Build history of the part. All positions in model axes, mm. Face numbers are marked on the shaded views. A direction names the side the tool comes from. Round coordinates to 2 decimals unless told otherwise and drop trailing zeros. Loops run counter-clockwise (first coordinate to the right, second up) from the corner with the lowest first, then second, coordinate; pieces in that order, holes last. Notation, with made-up numbers: (49.5, 10) -> (74.5, 10) arc R24 cw to (74.5, 28) -> close; hole circle Ø5 at (68, 1). An arc over 180 degrees is marked (long way). Put each result on its own line as item: value. Start each with the question number.
Item 1: Tool access for the marked faces 4, 5 and 6: list every direction of +Z, -Z, +X, -X, +Y, -Y with a clear straight run to the whole face (end or side of a thin tool).
Item 2: Flat gauge pins, fed straight in: pin 1 Ø8.5 at (x, z) = (0, 0) entering from +Y; pin 2 Ø3 at (x, z) = (4, 7) entering from +Y; pin 3 Ø1 at (x, z) = (-0.5, -1.5) entering from +Y. Where does each tip first touch, or does it go through?
Item 3: Cut at A-A, the plane y = -28. List the corners of the cut face in (x, z), plus the area to 3 significant figures.
Item 4: Pull direction X, two halves, no side cores. Call the marked faces 1, 2 and 3: +X half, -X half, draft (parallel to the pull), parting line (faces both ways), or undercut.
Item 5: Drill centre lines: probe 1 along X at (y, z) = (-32, 0); probe 2 along Y at (x, z) = (3.25, 5.5); probe 3 along Z at (x, y) = (0, -32.5). Where is each one in solid material? Low to high. Write a range as [from, to].
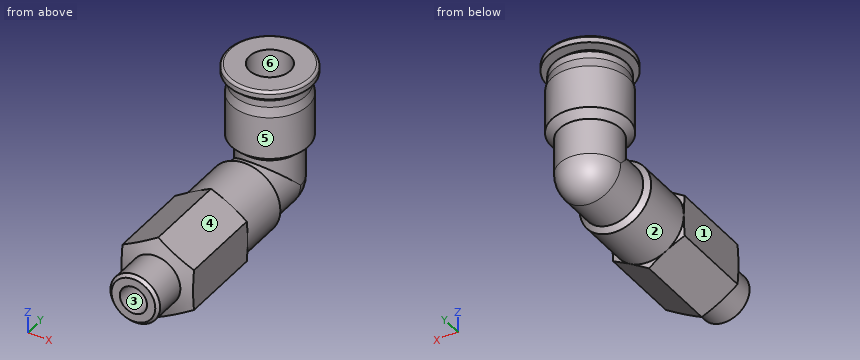
```python
from build123d import *

# Parameters (mm, degrees)
SKETCH_3_R          = 14
CUT_EXTRUDE_1_DEPTH = 21.4
SKETCH_5_W          = 2.666666667
SKETCH_5_H          = 42.8


with BuildPart() as part:
    # 草图1 → 旋转1 (revolve)
    with BuildSketch(Plane(origin=(0, 0, 0), x_dir=(0, 0, -1), z_dir=(1, 0, 0)), mode=Mode.PRIVATE) as revolve_1_sk:
        with BuildLine():
            Line((-22.5, 0), (-22.5, 7.75))
            ThreePointArc((-22.5, 7.75), (-22.353553391, 8.103553391), (-22, 8.25))
            Line((-22, 8.25), (-21, 8.25))
            Line((-21, 8.25), (-21, 6))
            Line((-21, 6), (-20.1, 6))
            Line((-20.1, 6), (-20.1, 6.925))
            ThreePointArc((-20.1, 6.925), (-20.041421356, 7.066421356), (-19.9, 7.125))
            Line((-19.9, 7.125), (-18.6, 7.125))
            Line((-18.6, 7.125), (-16.725, 7.5))
            Line((-16.725, 7.5), (-8.381856066, 7.5))
            Line((-8.381856066, 7.5), (-7.03125, 6))
            Line((-7.03125, 6), (0, 6))
            ThreePointArc((0, 6), (4.242640687, 4.242640687), (6, 0))
            Line((6, 0), (-22.5, 0))
        make_face()
    revolve(revolve_1_sk.sketch.rotate(Axis((0, 0, -6), (0, 0, 1)), 270), axis=Axis((0, 0, -6), (0, 0, 1)))

    # 草图2 → 旋转2 (revolve)
    with BuildSketch(Plane(origin=(0, 0, 0), x_dir=(0, 0, -1), z_dir=(1, 0, 0)), mode=Mode.PRIVATE) as revolve_2_sk:
        Polygon((0, -42.8), (-4.283, -42.8), (-4.864, -42.219), (-4.864, -35.872339475), (-8.082903769, -35.00983681), (-8.082903769, -18.47016319), (-7, -18.18), (-7, -7.931654044), (-6, -7.03125), (-6, 0), (0, 0), align=None)
    revolve(revolve_2_sk.sketch.rotate(Axis((0, 0, 0), (0, -1, 0)), 180), axis=Axis((0, 0, 0), (0, -1, 0)))

    # 草图3 → 切除-拉伸1 (cut)
    with BuildSketch(Plane(origin=(0, -35.3, 0), x_dir=(1, 0, 0), z_dir=(0, 1, 0))):
        Circle(SKETCH_3_R)
        Polygon((-7, 4.041451884), (-7, -4.041451884), (0, -8.082903769), (7, -4.041451884), (7, 4.041451884), (0, 8.082903769), align=None, mode=Mode.SUBTRACT)
    extrude(amount=CUT_EXTRUDE_1_DEPTH, mode=Mode.SUBTRACT)

    # 草图4 → 切除-旋转1 (revolve, cut)
    with BuildSketch(Plane(origin=(0, 0, 0), x_dir=(0, 0, -1), z_dir=(1, 0, 0)), mode=Mode.PRIVATE) as cut_revolve_1_sk:
        with BuildLine():
            Line((-22.5, 0), (-22.5, 4))
            Line((-22.5, 4), (0, 4))
            ThreePointArc((0, 4), (2.828427125, 2.828427125), (4, 0))
            Line((4, 0), (-22.5, 0))
        make_face()
    revolve(cut_revolve_1_sk.sketch.rotate(Axis((0, 0, -4), (0, 0, 1)), 270), axis=Axis((0, 0, -4), (0, 0, 1)), mode=Mode.SUBTRACT)

    # 草图5 → 切除-旋转2 (revolve, cut)
    with BuildSketch(Plane(origin=(0, 0, 0), x_dir=(0, 0, -1), z_dir=(1, 0, 0)), mode=Mode.PRIVATE) as cut_revolve_2_sk:
        with Locations((-1.333333334, -21.4)):
            Rectangle(SKETCH_5_W, SKETCH_5_H)
    revolve(cut_revolve_2_sk.sketch.rotate(Axis((0, 0, 0), (0, -1, 0)), 180), axis=Axis((0, 0, 0), (0, -1, 0)), mode=Mode.SUBTRACT)


solid = part.part
```
Reply:
1. face 4: +Z, +X, -Y
1. face 5: none
1. face 6: +Z
2. pin 1: stops at y = 6
2. pin 2: stops at y = 6.68
2. pin 3: stops at y = 5.9
3. outline: (-7, -4.04) -> (0, -8.08) -> (7, -4.04) -> (7, 4.04) -> (0, 8.08) -> (-7, 4.04) -> close; hole circle Ø5.33 at (0, 0)
3. area: 147 mm^2
4. face 1: -X half
4. face 2: parting line
4. face 3: undercut
5. probe 1: x = [-7, -2.67], [2.67, 7]
5. probe 2: y = [-35.46, -7.38], [-5.04, -2.33], [2.33, 5.04]
5. probe 3: z = [-8.08, -2.67], [2.67, 8.08]
